from build123d import *

# Parameters (mm, degrees)
SKETCH_1_W          = 12
SKETCH_1_H          = 12
SKETCH_1_W_2        = 8
SKETCH_1_H_2        = 8
EXTRUDE_1_DEPTH     = 275
SKETCH_3_R          = 2.05
SKETCH_3_R_2        = 2.1
CUT_EXTRUDE_2_DEPTH = 276.327078218


with BuildPart() as part:
    # 草图1 → 凸台-拉伸1 (new body)
    with BuildSketch(Plane(origin=(0, 0, 0), x_dir=(1, 0, 0), z_dir=(0, 1, 0))):
        Rectangle(SKETCH_1_W, SKETCH_1_H)
        Rectangle(SKETCH_1_W_2, SKETCH_1_H_2, mode=Mode.SUBTRACT)
    extrude(amount=EXTRUDE_1_DEPTH)

    # 草图3 → 切除-拉伸2 (cut, through all)
    with BuildSketch(Plane.ZY.offset(6)):
        with Locations((0, 265)):
            Circle(SKETCH_3_R)
        with Locations((0, 245)):
            Circle(SKETCH_3_R)
        with Locations((0, 220)):
            Circle(SKETCH_3_R)
        with Locations((0, 14.5)):
            Circle(SKETCH_3_R_2)
    extrude(amount=-CUT_EXTRUDE_2_DEPTH, mode=Mode.SUBTRACT)


solid = part.part
Input: part model. Units: mm. Frame: model coordinates. A direction names the side the tool comes from. Coordinates: 2 decimals unless noted, no trailing zeros. Order: outer loops, then holes, each group sorted by start corner. A loop starts at its lowest first (then second) coordinate and runs counter-clockwise, first axis right, second up.
1. Ray query, line 1 along Y through (x, z) = (-4.75, 0); line 2 along X through (y, z) = (52, -1.75). Return the intervals inside material, ascending.
Checked values:
line 1: y = 0 to 12.4, 16.6 to 217.95, 222.05 to 242.95, 247.05 to 262.95, 267.05 to 275
line 2: x = -6 to -4, 4 to 6
2. Cut plane A-A, the plane y = 93. Return loops of the section in (x, z).
Checked values:
outline: (-6, -6) - (6, -6) - (6, 6) - (-6, 6) - close; hole (-4, -4) - (4, -4) - (4, 4) - (-4, 4) - close
3. Cut plane C-C, the plane z = 0. Count the separate pieces of the cut face and the enclosed holes in it, plus the area to 3 significant figures.
Checked values:
separate pieces: 10
enclosed holes: 0
area: 1,030 mm2
4. Contact query for a flat-ended pin moving along its axis: P1, Ø3.5, axis at y = 265, z = 0, coming from the -X side. Output: stop coordinate, or through.
Checked values:
P1: passes through
5. Cut plane B-B, the plane x = -1.25. Return loops of the section in (y, z).
Checked values:
outline: (0, -6) - (275, -6) - (275, -4) - (0, -4) - close; (0, 4) - (275, 4) - (275, 6) - (0, 6) - close
6. Access query for faces 1 (the flat face through (0, 136, 4)), 2 (the flat face through (0, 136, 6)). Directions: +Z, -Z, +X, -X, +Y, -Y. A direction counts if a zero-diameter tool reaches every point of the face in a straight line with its end or side. Return the directions, or none.
Checked values:
face 1: +Y, -Y
face 2: +Z, +X, -X, +Y, -Y
7. Draft query along Z for faces 3 (the flat face through (6, 136, 0)), 4 (the cylindrical face through (-5.01, 16.27, 1.13)), 5 (the flat face through (0, 136, -6)). Return one class per face: +Z half, -Z half, draft (parallel to the pull), parting line (faces both ways), or undercut.
Checked values:
face 3: draft
face 4: undercut
face 5: -Z half
